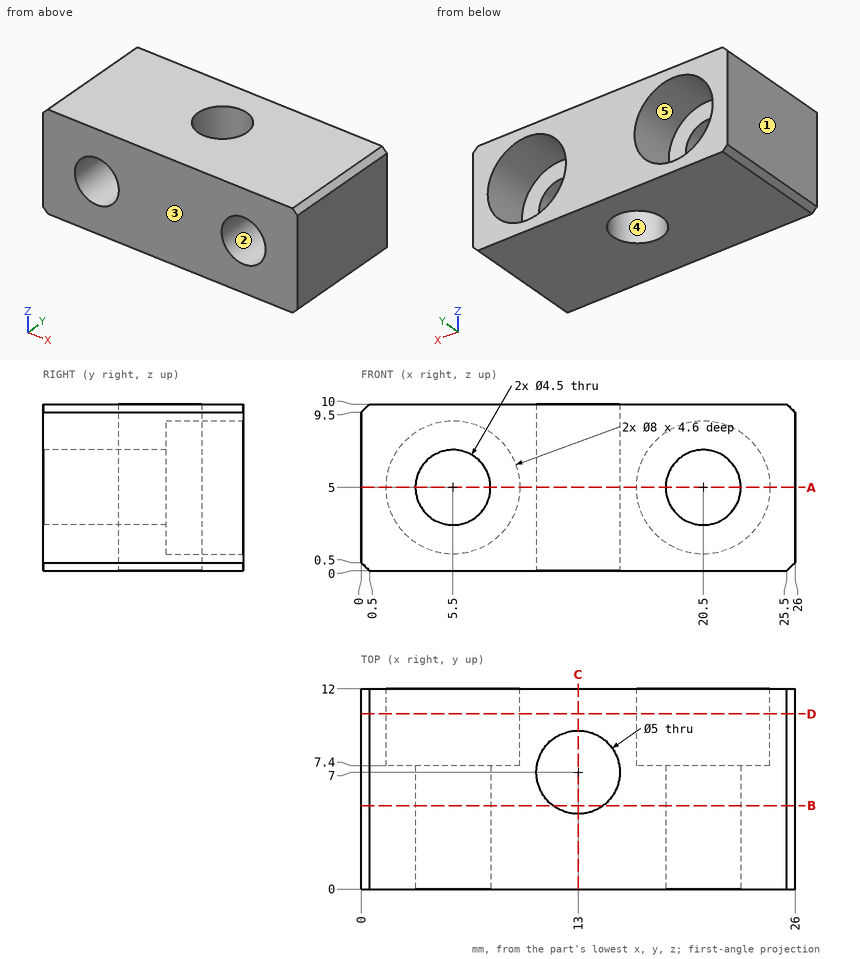
Drawing for the job (mm, zero at the part's lowest x, y, z). A direction names the side the tool comes from. Round coordinates to 2 decimals unless told otherwise and drop trailing zeros. Loops run counter-clockwise (first coordinate to the right, second up) from the corner with the lowest first, then second, coordinate; pieces in that order, holes last. Notation, with made-up numbers: (39.25, 81.25) -> (63.25, 81.25) arc R30 ccw to (63.25, 118.25) -> close; hole circle Ø5 at (25.5, -10.5). An arc over 180 degrees is marked (long way). Answer as CSV lines item,"result". Start each with the question number.
1) Slice it at D-D (y = 10.5). List the corners of the cut face in (x, z).
2) Slice it at B-B (y = 5). List the corners of the cut face in (x, z), plus the area to 3 significant figures.
3) Mould opens along X. For the marked faces 1, 2 and 3 say: +X half, -X half, draft (parallel to the pull), parting line (faces both ways), or undercut.
4) Slice it at A-A (z = 5). List the corners of the cut face in (x, y), plus the area to 3 significant figures.
5) Pin check, flat tips, straight feed: P1, Ø2.5, axis at x = 6, z = 4.5, coming from the +Y side; P2, Ø2.5, axis at x = 19.5, z = 6.5, coming from the +Y side. Stop position of each tip, or through.
6) Tool access for the marked faces 4 and 5: list every direction of +Z, -Z, +X, -X, +Y, -Y with a clear straight run to the whole face (end or side of a thin tool).
7) Slice it at C-C (x = 13). List the corners of the cut face in (y, z).
8) Probe line 1 along Y through (x, z) = (13, 5.5); line 2 along Z through (x, y) = (5.5, 3.5); line 3 along X through (y, z) = (6.5, 3.5). List the from-to ranges inside material, lowest first.
Filled in:
1,outline,"(0, 0.5) -> (0.5, 0) -> (25.5, 0) -> (26, 0.5) -> (26, 9.5) -> (25.5, 10) -> (0.5, 10) -> (0, 9.5) -> close; hole circle Ø8 at (5.5, 5); hole circle Ø8 at (20.5, 5)"
2,outline,"(0, 0.5) -> (0.5, 0) -> (11.5, 0) -> (11.5, 10) -> (0.5, 10) -> (0, 9.5) -> close; (14.5, 0) -> (25.5, 0) -> (26, 0.5) -> (26, 9.5) -> (25.5, 10) -> (14.5, 10) -> close; hole circle Ø4.5 at (5.5, 5); hole circle Ø4.5 at (20.5, 5)"
2,area,"198 mm2"
3,face 1,"-X half"
3,face 2,"undercut"
3,face 3,"draft"
4,outline,"(0, 0) -> (3.25, 0) -> (3.25, 7.4) -> (1.5, 7.4) -> (1.5, 12) -> (0, 12) -> close; (7.75, 0) -> (18.25, 0) -> (18.25, 7.4) -> (16.5, 7.4) -> (16.5, 12) -> (9.5, 12) -> (9.5, 7.4) -> (7.75, 7.4) -> close; (22.75, 0) -> (26, 0) -> (26, 12) -> (24.5, 12) -> (24.5, 7.4) -> (22.75, 7.4) -> close; hole circle Ø5 at (13, 7)"
4,area,"152 mm2"
5,P1,"passes through"
5,P2,"stops at y = 7.4"
6,face 4,"+Z, -Z"
6,face 5,"+Y"
7,outline,"(0, 0) -> (4.5, 0) -> (4.5, 10) -> (0, 10) -> close; (9.5, 0) -> (12, 0) -> (12, 10) -> (9.5, 10) -> close"
8,line 1,"y = 0 to 4.5, 9.5 to 12"
8,line 2,"z = 0 to 2.75, 7.25 to 10"
8,line 3,"x = 0 to 3.82, 7.18 to 10.55, 15.45 to 18.82, 22.18 to 26"
